The model under review builds one solid part; all positions refer to its coordinate system, in mm. A direction names the side the tool comes from. Give positions to 0.01 mm unless a question says otherwise; leave off trailing zeros. Order: outer loops, then holes, each group sorted by start corner. A loop starts at its lowest first (then second) coordinate and runs counter-clockwise, first axis right, second up. Notation, with made-up numbers: M 52,86 L 72,86 A18 cw 72,99 Z; hole C 3,71 d9. An arc over 180 degrees is marked long. One line per question, with ' | ' between items. Start each with the question number.
1. Wall thickness on L1, parallel to X at y = 3.25, z = 195; L2, parallel to Y at x = -217, z = 3; L3, parallel to X at y = 4.75, z = -23.5: over which ranges is each line inside the solid? List them lowest first.
2. The part is to be moulded in two halves that separate along X. For faces 1 (the face through (-50, -6, 50)), 2 (the face through (231.494, -1.07, -0.286)), 3 (the face through (10.55, -0.93, -239.77)), say which applies: +X half, -X half, draft (parallel to the pull), parting line (faces both ways), or undercut.
3. We need section D-D on x = -225. Write out the cut boundary in (y, z).
4. Insertion check: P1, Ø17, axis at x = 225, z = 0, coming from the +Y side; P2, Ø1.5, axis at x = -101.5, y = 3, coming from the -Z side. Each pin has a flat end and moves straight along its axis. Give the tip position at first contact, or say it passes through.
5. We need section B-B on x = 112.5. Write out the cut boundary in (y, z).
6. We need section A-A on z = 0. Write out the cut boundary in (x, y), then the cut area to 3 significant figures.
7. We need section C-C on y = -2.25. Write out the cut boundary in (x, z), then the cut area to 3 significant figures.
8. For faces 4 (the face through (113.35, -1.07, 188.41)), 5 (the face through (-1, 4, 212)), list the 3-axis set-ups (+Z, -Z, +X, -X, +Y, -Y) from which the entire face can be reached by the end or side of a thin tool; tool diameter is ignored.
```python
from build123d import *

# Parameters (mm, degrees)
SKETCH1_R                  = 240
SKETCH1_R_2                = 62.75
BOSS_EXTRUDE1_DEPTH        = 6
F_13_0_13_DIAMETER_HOLE1_D = 13
SKETCH4_OUTSIDE_W          = 617.786
SKETCH4_OUTSIDE_H          = 617.786
SKETCH4_OUTSIDE_R          = 210
CUT_EXTRUDE1_DEPTH         = 2


with BuildPart() as part:
    # Sketch1 → Boss-Extrude1 (new, symmetric)
    with BuildSketch(Plane(origin=(0, 0, 0), x_dir=(1, 0, 0), z_dir=(0, 1, 0))):
        with Locations(Location((0, 0, 0), (0, 0, 270))):
            Circle(SKETCH1_R)
        with Locations(Location((0, 0, 0), (0, 0, 270))):
            Circle(SKETCH1_R_2, mode=Mode.SUBTRACT)
    extrude(amount=BOSS_EXTRUDE1_DEPTH, both=True)

    # Ø13.0 (13) Diameter Hole1 (through all)
    with Locations(Plane(origin=(0, 6, 0), x_dir=(1, 0, 0), z_dir=(0, 1, 0))):
        with Locations((112.5, -194.855715851), (-112.5, -194.855715851), (-225, 0), (-112.5, 194.855715851), (112.5, 194.855715851), (225, 0)):
            Hole(F_13_0_13_DIAMETER_HOLE1_D / 2)

    # Sketch4 outside → Cut-Extrude1 (cut)
    with BuildSketch(Plane(origin=(0, 6, 0), x_dir=(1, 0, 0), z_dir=(0, 1, 0))):
        Rectangle(SKETCH4_OUTSIDE_W, SKETCH4_OUTSIDE_H)
        with Locations(Location((0, 0, 0), (0, 0, 270))):
            Circle(SKETCH4_OUTSIDE_R, mode=Mode.SUBTRACT)
    extrude(amount=-CUT_EXTRUDE1_DEPTH, mode=Mode.SUBTRACT)


solid = part.part
```
Entries:
1) L1: x = -139.91 to -119, -106 to 106, 119 to 139.91 | L2: y = -6 to 4 | L3: x = -208.68 to -58.18, 58.18 to 208.68
2) face 1: draft | face 2: undercut | face 3: parting line
3) outline: M -6,-83.52 L 4,-83.52 L 4,-6.5 L -6,-6.5 Z; M -6,6.5 L 4,6.5 L 4,83.52 L -6,83.52 Z
4) P1: stops at y = 4 | P2: stops at z = -217.83
5) outline: M -6,-212 L 4,-212 L 4,-201.36 L -6,-201.36 Z; M -6,-188.36 L 4,-188.36 L 4,-177.32 L 6,-177.32 L 6,177.32 L 4,177.32 L 4,188.36 L -6,188.36 Z; M -6,201.36 L 4,201.36 L 4,212 L -6,212 Z
6) outline: M -240,-6 L -231.5,-6 L -231.5,4 L -240,4 Z; M -218.5,-6 L -62.75,-6 L -62.75,6 L -210,6 L -210,4 L -218.5,4 Z; M 62.75,-6 L 218.5,-6 L 218.5,4 L 210,4 L 210,6 L 62.75,6 Z; M 231.5,-6 L 240,-6 L 240,4 L 231.5,4 Z | area: 3,870 mm^2
7) outline: C 0,0 d480; hole C -225,0 d13; hole C -112.5,-194.86 d13; hole C -112.5,194.86 d13; hole C 0,0 d125.5; hole C 112.5,-194.86 d13; hole C 112.5,194.86 d13; hole C 225,0 d13 | area: 168,000 mm^2
8) face 4: +Y, -Y | face 5: +Y
